Here's the drawing with two shaded views (mm, measured from the low corner). I have some questions. Give positions to 0.01 mm unless a question says otherwise; leave off trailing zeros. Loops run counter-clockwise (first coordinate to the right, second up) from the corner with the lowest first, then second, coordinate; pieces in that order, holes last. Notation, with made-up numbers: (32, 86.25) -> (50, 86.25) arc R27 ccw to (50, 107.25) -> close; hole circle Ø7 at (-23.75, -23.5). An arc over 180 degrees is marked (long way). Put each result on its own line as item: value.
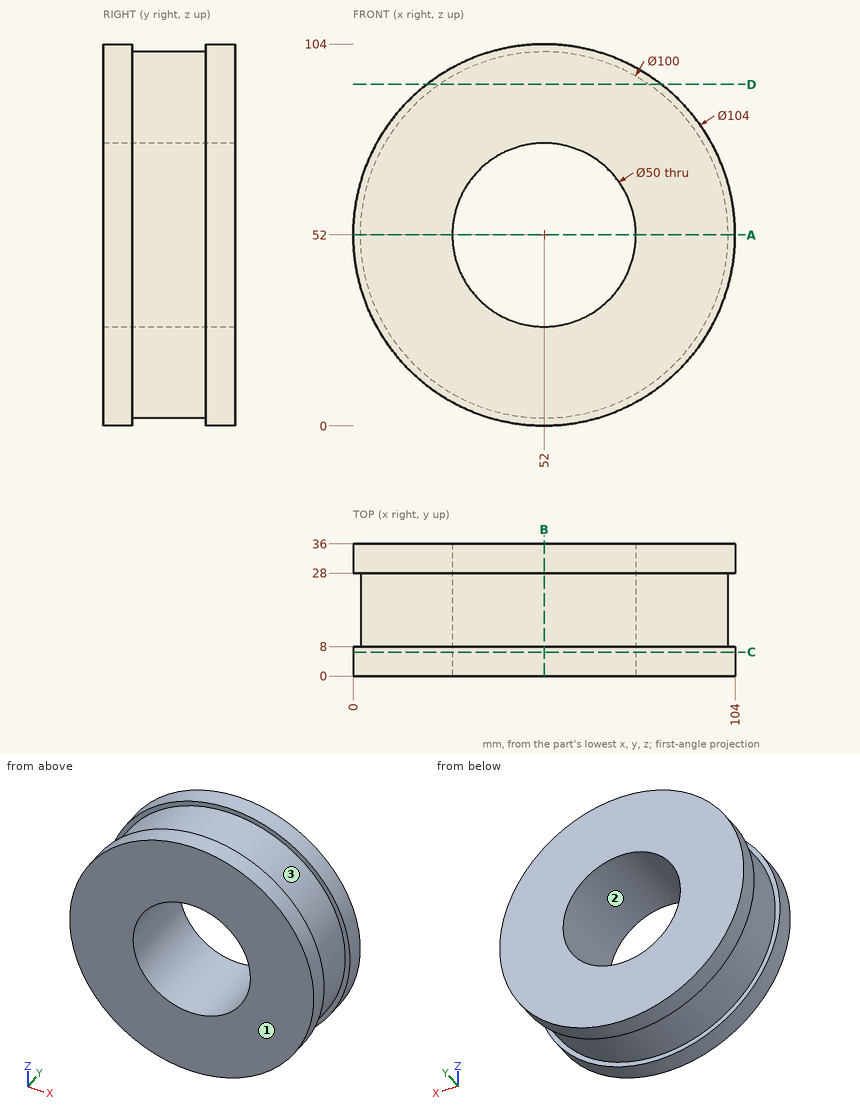
1. If we section it at C-C (y = 6.5): List the corners of the cut face in (x, z) for me, then the cut area to 3 significant figures.
Recorded:
outline: circle Ø104 at (52, 52); hole circle Ø50 at (52, 52)
area: 6,530 mm^2
2. If we section it at D-D (z = 93): List the corners of the cut face in (x, y) for me, then the cut area to 3 significant figures.
Recorded:
outline: (20.02, 0) -> (83.98, 0) -> (83.98, 8) -> (80.62, 8) -> (80.62, 28) -> (83.98, 28) -> (83.98, 36) -> (20.02, 36) -> (20.02, 28) -> (23.38, 28) -> (23.38, 8) -> (20.02, 8) -> close
area: 2,170 mm^2
3. Thinking about a two-plate mould opening in Z: for the marked faces 1, 2 and 3, which applies, pulls with the +Z half, pulls with the -Z half, needs draft (parallel to the pull), parting line crosses it, or undercut?
Recorded:
face 1: needs draft
face 2: undercut
face 3: parting line crosses it
4. I'm going to push flat-ended pins straight in: pin 1 (12 mm diameter, centred on x = 81, y = 13, fed in from +Z); pin 2 (1 mm diameter, centred on y = 10.5, z = 71, fed in from -X); pin 3 (1.5 mm diameter, centred on x = 19, y = 22, fed in from +Z). Where does each tip first touch, or does it pass through?
Recorded:
pin 1: stops at z = 97.21
pin 2: stops at x = 5.55
pin 3: stops at z = 90.21
5. If we section it at B-B (x = 52): List the corners of the cut face in (y, z) for me, then the cut area to 3 significant figures.
Recorded:
outline: (0, 0) -> (8, 0) -> (8, 2) -> (28, 2) -> (28, 0) -> (36, 0) -> (36, 27) -> (0, 27) -> close; (0, 77) -> (36, 77) -> (36, 104) -> (28, 104) -> (28, 102) -> (8, 102) -> (8, 104) -> (0, 104) -> close
area: 1,860 mm^2
6. I need wall thicknesses on line 1 (X direction, y = 13.5, z = 52); line 2 (X direction, y = 28.5, z = 52); line 3 (Z direction, x = 59.5, y = 31). Which ranges of each line are inside material? Lowest first, please.
Recorded:
line 1: x = 2 to 27, 77 to 102
line 2: x = 0 to 27, 77 to 104
line 3: z = 0.54 to 28.15, 75.85 to 103.46
7. If we section it at A-A (z = 52): List the corners of the cut face in (x, y) for me, then the cut area to 3 significant figures.
Recorded:
outline: (0, 0) -> (27, 0) -> (27, 36) -> (0, 36) -> (0, 28) -> (2, 28) -> (2, 8) -> (0, 8) -> close; (77, 0) -> (104, 0) -> (104, 8) -> (102, 8) -> (102, 28) -> (104, 28) -> (104, 36) -> (77, 36) -> close
area: 1,860 mm^2
